```python
from build123d import *

# Parameters (mm, degrees)
SKETCH1_R                                            = 21
BOSS_EXTRUDE1_DEPTH                                  = 10
SKETCH2_W                                            = 9
SKETCH2_H                                            = 18.909216571
CUT_EXTRUDE1_DEPTH                                   = 12
FILLET1_R                                            = 1
CIRPATTERN1_COUNT                                    = 3
FILLET1_OF_CIRPATTERN1_R                             = 1
CBORE_FOR_M2_5_HEX_SOCKET_HEAD_CAP_SCREW_D           = 2.9
CBORE_FOR_M2_5_HEX_SOCKET_HEAD_CAP_SCREW_CBORE_D     = 5.5
CBORE_FOR_M2_5_HEX_SOCKET_HEAD_CAP_SCREW_CBORE_DEPTH = 2.9
CIRPATTERN2_COUNT                                    = 3
CUT_EXTRUDE2_DEPTH                                   = 32.336879232
FILLET2_R                                            = 1
CIRPATTERN3_COUNT                                    = 3
FILLET2_OF_CIRPATTERN3_R                             = 1
SKETCH7_R                                            = 5
CUT_EXTRUDE4_DEPTH                                   = 2.5


with BuildPart() as part:
    # Sketch1 → Boss-Extrude1 (new body)
    with BuildSketch(Plane.XY):
        Circle(SKETCH1_R)
    extrude(amount=BOSS_EXTRUDE1_DEPTH)

    # Sketch2 → Cut-Extrude1 (cut)
    with BuildSketch(Plane.XY.offset(10)):
        with Locations((0, 15.954608286)):
            Rectangle(SKETCH2_W, SKETCH2_H)
    cut_extrude1 = extrude(amount=-CUT_EXTRUDE1_DEPTH, mode=Mode.SUBTRACT)

    # Fillet1
    fillet1_edges = [part.edges().sort_by_distance(p)[0] for p in [
        (-4.5, 20.512191497, 5),
        (-4.5, 6.5, 5),
        (4.5, 20.512191497, 5),
        (4.5, 6.5, 5),
    ]]
    fillet(fillet1_edges, radius=FILLET1_R)

    # CirPattern1: Cut-Extrude1 ×3 about axis
    cirpattern1_axis = Axis((0, 0, 0), (0, 0, 1))
    for i in range(1, CIRPATTERN1_COUNT):
        add(cut_extrude1.rotate(cirpattern1_axis, i * 360 / CIRPATTERN1_COUNT), mode=Mode.SUBTRACT)

    # Fillet1 of CirPattern1
    fillet1_of_cirpattern1_edges = [part.edges().sort_by_distance(p)[0] for p in [
        (-15.514078923, -14.153210065, 5),
        (-3.379165125, -7.147114317, 5),
        (-20.014078923, -6.358981431, 5),
        (-7.879165125, 0.647114317, 5),
        (20.014078923, -6.358981431, 5),
        (7.879165125, 0.647114317, 5),
        (15.514078923, -14.153210065, 5),
        (3.379165125, -7.147114317, 5),
    ]]
    fillet(fillet1_of_cirpattern1_edges, radius=FILLET1_OF_CIRPATTERN1_R)

    # CBORE for M2.5 Hex Socket Head Cap Screw1 (through all)
    with Locations(Plane.XY.offset(10)):
        with Locations((0, -9)):
            cbore_for_m2_5_hex_socket_head_cap_screw = CounterBoreHole(CBORE_FOR_M2_5_HEX_SOCKET_HEAD_CAP_SCREW_D / 2, CBORE_FOR_M2_5_HEX_SOCKET_HEAD_CAP_SCREW_CBORE_D / 2, CBORE_FOR_M2_5_HEX_SOCKET_HEAD_CAP_SCREW_CBORE_DEPTH)

    # CirPattern2: CBORE for M2.5 Hex Socket Head Cap Screw1 ×3 about axis
    cirpattern2_axis = Axis((0, 0, 0), (0, 0, 1))
    for i in range(1, CIRPATTERN2_COUNT):
        add(cbore_for_m2_5_hex_socket_head_cap_screw.rotate(cirpattern2_axis, i * 360 / CIRPATTERN2_COUNT), mode=Mode.SUBTRACT)

    # Sketch5 → Cut-Extrude2 (cut, through all)
    with BuildSketch(Plane.XY.offset(10)):
        with BuildLine():
            Line((4, -17), (4, -24.000575883))
            ThreePointArc((4, -24.000575883), (0, -28.000575883), (-4, -24.000575883))
            Line((-4, -24.000575883), (-4, -17))
            ThreePointArc((-4, -17), (0, -13), (4, -17))
        make_face()
    cut_extrude2 = extrude(amount=-CUT_EXTRUDE2_DEPTH, mode=Mode.SUBTRACT)

    # Fillet2
    fillet2_edges = [part.edges().sort_by_distance(p)[0] for p in [
        (4, -20.615528128, 5),
        (-4, -20.615528128, 5),
    ]]
    fillet(fillet2_edges, radius=FILLET2_R)

    # CirPattern3: Cut-Extrude2 ×3 about axis
    cirpattern3_axis = Axis((0, 0, 0), (0, 0, 1))
    for i in range(1, CIRPATTERN3_COUNT):
        add(cut_extrude2.rotate(cirpattern3_axis, i * 360 / CIRPATTERN3_COUNT), mode=Mode.SUBTRACT)

    # Fillet2 of CirPattern3
    fillet2_of_cirpattern3_edges = [part.edges().sort_by_distance(p)[0] for p in [
        (15.853571071, 13.771865679, 5),
        (19.853571071, 6.843662449, 5),
        (-19.853571071, 6.843662449, 5),
        (-15.853571071, 13.771865679, 5),
    ]]
    fillet(fillet2_of_cirpattern3_edges, radius=FILLET2_OF_CIRPATTERN3_R)

    # Sketch7 → Cut-Extrude4 (cut)
    with BuildSketch(Plane.XY.offset(10)):
        Circle(SKETCH7_R)
    extrude(amount=-CUT_EXTRUDE4_DEPTH, mode=Mode.SUBTRACT)


solid = part.part
```
Verification items for the finished model (mm, model axes). A direction names the side the tool comes from. Give positions to 0.01 mm unless a question says otherwise; leave off trailing zeros. Order: outer loops, then holes, each group sorted by start corner. A loop starts at its lowest first (then second) coordinate and runs counter-clockwise, first axis right, second up. Notation, with made-up numbers: (-12.75, 40.5) -> (21.25, 40.5) arc R22 ccw to (21.25, 70.5) -> close; hole circle Ø2 at (47, -27). An arc over 180 degrees is marked (long way). Use a Markdown table: item, result.
1) Section check C-C, the plane y = -4.5. Record the boundary of the cut face in (x, z), then the cut area to 3 significant figures.
Results:
| item | result |
|---|---|
| outline | (-20.51, 0) -> (-16.79, 0) -> (-16.79, 10) -> (-20.51, 10) -> close; (-4.91, 0) -> (4.91, 0) -> (4.91, 10) -> (2.18, 10) -> (2.18, 7.5) -> (-2.18, 7.5) -> (-2.18, 10) -> (-4.91, 10) -> close; (16.79, 0) -> (20.51, 0) -> (20.51, 10) -> (16.79, 10) -> close |
| area | 162 mm² |
2) Tool access check on faces 1 (the flat face through (8.2, 6.1, 7.1)), 2 (the flat face through (-4.5, 13, 5)), 3 (the cylindrical face through (11.303, 6.424, 5.07)), 4 (the cylindrical face through (-15.26, 13.86, 4.93)), 5 (the flat face through (13.732, 12.547, 5.07)). Record the directions out of +Z, -Z, +X, -X, +Y, -Y that give a thin tool (end or side, any length) a straight path to the whole face; none if there is none.
Results:
| item | result |
|---|---|
| face 1 | +Z |
| face 2 | +Z, -Z, +Y |
| face 3 | +Z, -Z |
| face 4 | +Z, -Z, -X |
| face 5 | +Z, -Z, +X |
3) Section check A-A, the plane y = 8.5. Record the boundary of the cut face in (x, z), then the cut area to 3 significant figures.
Results:
| item | result |
|---|---|
| outline | (-10.72, 0) -> (-4.5, 0) -> (-4.5, 10) -> (-10.72, 10) -> close; (4.5, 0) -> (10.72, 0) -> (10.72, 10) -> (4.5, 10) -> close |
| area | 124 mm² |
4) Section check B-B, the plane x = 0. Record the boundary of the cut face in (y, z), then the cut area to 3 significant figures.
Results:
| item | result |
|---|---|
| outline | (-13, 0) -> (-10.45, 0) -> (-10.45, 7.1) -> (-11.75, 7.1) -> (-11.75, 10) -> (-13, 10) -> close; (-7.55, 0) -> (6.5, 0) -> (6.5, 10) -> (5, 10) -> (5, 7.5) -> (-5, 7.5) -> (-5, 10) -> (-6.25, 10) -> (-6.25, 7.1) -> (-7.55, 7.1) -> close |
| area | 133 mm² |
5) Material ranges on probe 1 along Y at (x, z) = (0, 9.1); probe 2 along X at (y, z) = (-3, 8.5); probe 3 along X at (y, z) = (3, 8), recorded low to high.
Results:
| item | result |
|---|---|
| probe 1 | -13 to -11.75, -6.25 to -5, 5 to 6.5 |
| probe 2 | -20.78 to -14.2, -5.77 to -4, 4 to 5.77, 14.2 to 20.78 |
| probe 3 | -20.78 to -10.1, -5.49 to -4, 4 to 5.49, 10.1 to 20.78 |
6) Mould release check, pull along Y, two halves, no side actions. Record for faces 6 (the flat face through (4, -4, 10)), 7 (the flat face through (0, 6.5, 5)), 8 (the flat face through (0, 0, 7.5)): pulls with the +Y half, pulls with the -Y half, needs draft (parallel to the pull), parting line crosses it, or undercut.
Results:
| item | result |
|---|---|
| face 6 | needs draft |
| face 7 | pulls with the +Y half |
| face 8 | undercut |
7) Section check D-D, the plane y = -9. Record the boundary of the cut face in (x, z), then the cut area to 3 significant figures.
Results:
| item | result |
|---|---|
| outline | (-6.59, 0) -> (-1.45, 0) -> (-1.45, 7.1) -> (-2.75, 7.1) -> (-2.75, 10) -> (-6.59, 10) -> close; (1.45, 0) -> (6.59, 0) -> (6.59, 10) -> (2.75, 10) -> (2.75, 7.1) -> (1.45, 7.1) -> close |
| area | 95.2 mm² |
8) Depth check by flat-ended pin: pin 1 Ø13 at (x, y) = (0, 0) entering from -Z; pin 2 Ø4 at (y, z) = (-10, 6.5) entering from +X; pin 3 Ø3 at (y, z) = (3, 6.5) entering from -X; pin 4 Ø1.6 at (x, y) = (-1, -10) entering from +Z. Enter the tip coordinate at first touch or a pass-through.
Results:
| item | result |
|---|---|
| pin 1 | z = 0 |
| pin 2 | x = 11.78 |
| pin 3 | x = -20.95 |
| pin 4 | z = 7.1 |
